The listing builds one solid part. Answer for the finished solid, in the listing's coordinates (mm). A direction names the side the tool comes from. Round coordinates to 2 decimals unless told otherwise and drop trailing zeros. Write each loop counter-clockwise with the first axis right and the second up, starting at its lowest first coordinate (ties: lowest second). Pieces come first, ordered by that corner, then holes.
from build123d import *

# Parameters (mm, degrees)
BASE_PLATE_DEPTH         = 1
STANDOFF_WEB_SKETCH_W    = 4
STANDOFF_WEB_SKETCH_H    = 1
STANDOFF_WEB_4MM_DEPTH   = 4
FORK_LUG_SKETCH_W        = 4
FORK_LUG_SKETCH_H        = 9
FORK_LUG_DEPTH           = 1
LUG_END_FILLETS_R1_5_R   = 1.5
LUG_PIN_HOLES_SKETCH_R   = 0.75
LUG_PIN_HOLES_SKETCH_R_2 = 0.749568333
LUG_PIN_HOLES_DEPTH      = 1


with BuildPart() as part:
    # Base Plate Sketch → Base Plate (new body)
    with BuildSketch(Plane.XY):
        with BuildLine():
            Line((0, 0), (6, 0))
            Line((6, 0), (6, 1))
            Line((6, 1), (5, 1))
            ThreePointArc((5, 1), (4, 2), (5, 3))
            Line((5, 3), (6, 3))
            Line((6, 3), (6, 6))
            Line((6, 6), (5, 6))
            ThreePointArc((5, 6), (4, 7), (5, 8))
            Line((5, 8), (6, 8))
            Line((6, 8), (6, 9))
            Line((6, 9), (0, 9))
            Line((0, 9), (0, 8))
            Line((0, 8), (1, 8))
            ThreePointArc((1, 8), (2, 7), (1, 6))
            Line((1, 6), (0, 6))
            Line((0, 6), (0, 3))
            Line((0, 3), (1, 3))
            ThreePointArc((1, 3), (2, 2), (1, 1))
            Line((1, 1), (0, 1))
            Line((0, 1), (0, 0))
        make_face()
    extrude(amount=BASE_PLATE_DEPTH)

    # Standoff Web Sketch → Standoff Web 4mm (add)
    with BuildSketch(Plane(origin=(0, 0, 0), x_dir=(-1, 0, 0), z_dir=(0, 0, -1))):
        with Locations((-3, 4.5)):
            Rectangle(STANDOFF_WEB_SKETCH_W, STANDOFF_WEB_SKETCH_H)
    extrude(amount=STANDOFF_WEB_4MM_DEPTH)

    # Fork Lug Sketch → Fork Lug (add)
    with BuildSketch(Plane(origin=(0, 0, -4), x_dir=(-1, 0, 0), z_dir=(0, 0, -1))):
        with Locations((-3, 4.5)):
            Rectangle(FORK_LUG_SKETCH_W, FORK_LUG_SKETCH_H)
    extrude(amount=FORK_LUG_DEPTH)

    # Lug End Fillets R1.5
    lug_end_fillets_r1_5_edges = [part.edges().sort_by_distance(p)[0] for p in [
        (1, 0, -4.5),
        (1, 9, -4.5),
        (5, 9, -4.5),
        (5, 0, -4.5),
    ]]
    fillet(lug_end_fillets_r1_5_edges, radius=LUG_END_FILLETS_R1_5_R)

    # Lug Pin Holes Sketch → Lug Pin Holes (cut)
    with BuildSketch(Plane(origin=(0, 0, -5), x_dir=(-1, 0, 0), z_dir=(0, 0, -1))):
        with Locations((-3, 7.5)):
            Circle(LUG_PIN_HOLES_SKETCH_R)
        with Locations((-3, 1.5)):
            Circle(LUG_PIN_HOLES_SKETCH_R_2)
    extrude(amount=-LUG_PIN_HOLES_DEPTH, mode=Mode.SUBTRACT)


solid = part.part
1. Section B-B on y = 2 is taken. Determine the outline of the cut face in (x, z), plus the area to 3 significant figures.
Geometry says:
outline: (1, -5) - (2.44, -5) - (2.44, -4) - (1, -4) - close; (2, 0) - (4, 0) - (4, 1) - (2, 1) - close; (3.56, -5) - (5, -5) - (5, -4) - (3.56, -4) - close
area: 4.88 mm2
2. Section A-A on x = 5.3 is taken. Determine the outline of the cut face in (y, z).
Geometry says:
outline: (0, 0) - (1, 0) - (1, 1) - (0, 1) - close; (3, 0) - (6, 0) - (6, 1) - (3, 1) - close; (8, 0) - (9, 0) - (9, 1) - (8, 1) - close
3. Straight lines are drawn through the part: line 1 along Y through (x, z) = (3, -4.5); line 2 along Z through (x, y) = (4, 6); line 3 along Z through (x, y) = (1.6, 1.5). For each, find the intervals that lie inside material, in ascending order.
Geometry says:
line 1: y = 0 to 0.75, 2.25 to 6.75, 8.25 to 9
line 2: z = -5 to -4, 0 to 1
line 3: z = -5 to -4
4. A tool of negligible diameter and unlimited length cuts with its end or side. For faces 1 (the face through (1.45, 8.57, -4.51)), 2 (the face through (1.45, 0.43, -4.51)), 3 (the face through (5.5, 3, 0.5)), from which of +Z, -Z, +X, -X, +Y, -Y can it reach the whole face along a straight path? Write none if from no direction.
Geometry says:
face 1: -Z, -X, +Y
face 2: -Z, -X, -Y
face 3: +Z, -Z, +X
5. Section C-C on z = -4.3 is taken. Determine the outline of the cut face in (x, y).
Geometry says:
outline: (1, 1.5) arc R1.5 ccw to (2.5, 0) - (3.5, 0) arc R1.5 ccw to (5, 1.5) - (5, 7.5) arc R1.5 ccw to (3.5, 9) - (2.5, 9) arc R1.5 ccw to (1, 7.5) - close; hole circle Ø1.5 at (3, 1.5); hole circle Ø1.5 at (3, 7.5)
6. For a pull along Y with two mould halves and no side action, classify faces 4 (the face through (3, 9, -4.5)), 5 (the face through (5.5, 8, 0.5)), 6 (the face through (3.75, 1.53, -4.51)), 7 (the face through (6, 0.5, 0.5)) as released by +Y, released by -Y, zero draft, split by the parting line, or undercut.
Geometry says:
face 4: released by +Y
face 5: undercut
face 6: undercut
face 7: zero draft
7. Given pin 1 (1.1 mm diameter, centred on x = 5.5, z = 0.5, fed in from -Y); pin 2 (3 mm diameter, centred on y = 2, z = -4, fed in from -X), each flat-ended and moving along its own axis, determine where each tip first touches the part or whether it passes through.
Geometry says:
pin 1: stops at y = 0
pin 2: stops at x = 1
8. Section D-D on x = 3 is taken. Determine the outline of the cut face in (y, z), plus the area to 3 significant figures.
Geometry says:
outline: (0, -5) - (0.75, -5) - (0.75, -4) - (0, -4) - close; (0, 0) - (4, 0) - (4, -4) - (2.25, -4) - (2.25, -5) - (6.75, -5) - (6.75, -4) - (5, -4) - (5, 0) - (9, 0) - (9, 1) - (0, 1) - close; (8.25, -5) - (9, -5) - (9, -4) - (8.25, -4) - close
area: 19.0 mm2
